from build123d import *

# Parameters (mm, degrees)
SKETCH_1_W      = 50
SKETCH_1_H      = 50
SKETCH_1_W_2    = 44
SKETCH_1_H_2    = 44
EXTRUDE_1_DEPTH = 520


with BuildPart() as part:
    # 草图1 → 凸台-拉伸1 (new body)
    with BuildSketch(Plane.XY):
        with Locations((25, 25)):
            Rectangle(SKETCH_1_W, SKETCH_1_H)
        with Locations((25, 25)):
            Rectangle(SKETCH_1_W_2, SKETCH_1_H_2, mode=Mode.SUBTRACT)
    extrude(amount=EXTRUDE_1_DEPTH)


solid = part.part
Model file for the job. Use its own axes, mm. A direction names the side the tool comes from. Coordinates: 2 decimals unless noted, no trailing zeros. Write each loop counter-clockwise with the first axis right and the second up, starting at its lowest first coordinate (ties: lowest second). Pieces come first, ordered by that corner, then holes. Notation, with made-up numbers: (-39.75, -38) -> (-8.75, -38) arc R20 ccw to (-8.75, -32) -> close; hole circle Ø1 at (53, 57.25). An arc over 180 degrees is marked (long way). One line per item, written item: value. Start each with the question number.
1) Probe probe 1 along X at (y, z) = (46.5, 390). List the from-to ranges inside material, lowest first.
2) Pull direction Y, two halves, no side cores. Call faces 1 (the face through (25, 50, 256)), 2 (the face through (47, 25, 256)), 3 (the face through (2.7, 25.1, 0)), 4 (the face through (25, 3, 256)): +Y half, -Y half, draft (parallel to the pull), parting line (faces both ways), or undercut.
3) Slice it at A-A on z = 438.5. Write the cut outline in (x, y).
4) Slice it at B-B on y = 25. Write the cut outline in (x, z).
5) Which spindle directions (+Z, -Z, +X, -X, +Y, -Y) get a long thin tool onto all of the face, cutting with end or side? Do faces 5 (the face through (3, 25, 256)), 6 (the face through (50, 25, 256)). Say none if no direction does.
Answers follow:
1. probe 1: 0 to 3, 47 to 50
2. face 1: +Y half
2. face 2: undercut
2. face 3: draft
2. face 4: undercut
3. outline: (0, 0) -> (50, 0) -> (50, 50) -> (0, 50) -> close; hole (3, 3) -> (47, 3) -> (47, 47) -> (3, 47) -> close
4. outline: (0, 0) -> (3, 0) -> (3, 520) -> (0, 520) -> close; (47, 0) -> (50, 0) -> (50, 520) -> (47, 520) -> close
5. face 5: +Z, -Z
5. face 6: +Z, -Z, +X, +Y, -Y
